```python
from build123d import *

# Parameters (mm, degrees)
BOSS_EXTRUDE1_DEPTH = 20
CHAMFER1_SIZE       = 3
M6_TAPPED_HOLE1_D   = 5


with BuildPart() as part:
    # Sketch1 → Boss-Extrude1 (new body)
    with BuildSketch(Plane.XY):
        with BuildLine():
            Line((-7.5, -231.178372691), (-7.5, -247.778372691))
            Line((-7.5, -247.778372691), (7.5, -247.778372691))
            Line((7.5, -247.778372691), (7.5, -231.178372691))
            ThreePointArc((7.5, -231.178372691), (0, -231.3), (-7.5, -231.178372691))
        make_face()
    extrude(amount=BOSS_EXTRUDE1_DEPTH)

    # Chamfer1
    chamfer1_edges = [part.edges().sort_by_distance(p)[0] for p in [
        (7.5, -247.778372691, 10),
        (-7.5, -247.778372691, 10),
    ]]
    chamfer(chamfer1_edges, length=CHAMFER1_SIZE)

    # M6 Tapped Hole1 (through all)
    with Locations(Plane.XY.offset(20)):
        with Locations((0, -239.178372691)):
            Hole(M6_TAPPED_HOLE1_D / 2)


solid = part.part
```
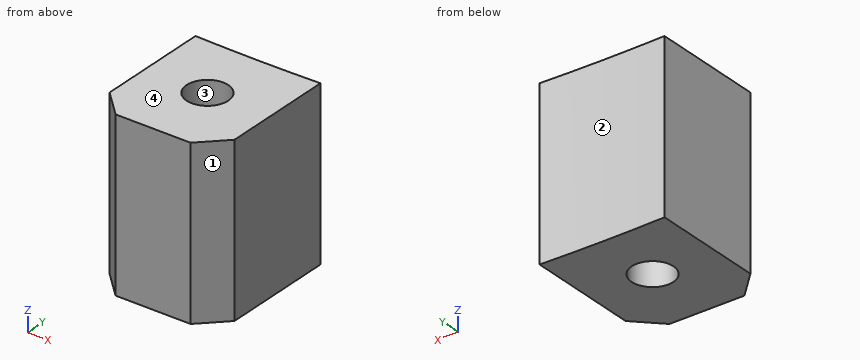
Can you work these out from the model? Positions are in its coordinate system, mm. Face numbers are marked on the shaded views. Give positions to 0.01 mm unless a question says otherwise; leave off trailing zeros. Loops run counter-clockwise (first coordinate to the right, second up) from the corner with the lowest first, then second, coordinate; pieces in that order, holes last. Notation, with made-up numbers: M 1,9.25 L 25,9.25 A36 ccw 25,46.25 Z; hole C -29,-3.5 d1. An arc over 180 degrees is marked long. One line per item, written item: value.
(1) We'd pull the mould along X, two halves only. Please class the marked faces 1, 2, 3 and 4: released by +X, released by -X, zero draft, split by the parting line, or undercut.
Returned:
face 1: released by +X
face 2: undercut
face 3: undercut
face 4: zero draft
(2) Suppose I cut it at D-D on y = -246.25. List the corners of the cut face in (x, z) for me.
Returned:
outline: M -6.03,0 L 6.03,0 L 6.03,20 L -6.03,20 Z
(3) Suppose I cut it at C-C on x = 1.75. List the corners of the cut face in (y, z) for me, plus the area to 3 significant figures.
Returned:
outline: M -247.78,0 L -240.96,0 L -240.96,20 L -247.78,20 Z; M -237.39,0 L -231.29,0 L -231.29,20 L -237.39,20 Z
area: 258 mm^2
(4) I need wall thicknesses on line 1 (Y direction, x = 0.5, z = 11.5); line 2 (Y direction, x = -3.75, z = 16.5); line 3 (Y direction, x = 6.75, z = 4.5). Which ranges of each line are inside material? Lowest first, please.
Returned:
line 1: -247.78 to -241.63, -236.73 to -231.3
line 2: -247.78 to -231.27
line 3: -245.53 to -231.2
(5) Suppose I cut it at B-B on z = 9. List the corners of the cut face in (x, y) for me, plus the area to 3 significant figures.
Returned:
outline: M -7.5,-244.78 L -4.5,-247.78 L 4.5,-247.78 L 7.5,-244.78 L 7.5,-231.18 A231.3 cw -7.5,-231.18 Z; hole C 0,-239.18 d5
area: 219 mm^2
(6) Suppose I cut it at A-A on x = 0. List the corners of the cut face in (y, z) for me.
Returned:
outline: M -247.78,0 L -241.68,0 L -241.68,20 L -247.78,20 Z; M -236.68,0 L -231.3,0 L -231.3,20 L -236.68,20 Z
(7) Will these pins go through, and if not, where does the flat tip stop? pin 1 (5 mm diameter, centred on x = 4.5, y = -238, fed in from -Z); pin 2 (1 mm diameter, centred on x = -4.5, z = 6, fed in from +Y).
Returned:
pin 1: z = 0
pin 2: y = -231.25
